```python
from build123d import *

# Parameters (mm, degrees)
SKETCH1_R           = 6.5
SKETCH1_R_2         = 3
BOSS_EXTRUDE1_DEPTH = 5
SKETCH2_R           = 10
BOSS_EXTRUDE2_DEPTH = 10
SKETCH3_W           = 22
SKETCH3_H           = 22
BOSS_EXTRUDE3_DEPTH = 3
FILLET1_R           = 3
SKETCH4_R           = 1.5
CUT_EXTRUDE1_DEPTH  = 3


with BuildPart() as part:
    # Sketch1 → Boss-Extrude1 (new body)
    with BuildSketch(Plane.XY):
        with Locations((-148.746139417, 0)):
            Circle(SKETCH1_R)
        with Locations((-148.746139417, 0)):
            Circle(SKETCH1_R_2, mode=Mode.SUBTRACT)
    extrude(amount=BOSS_EXTRUDE1_DEPTH)

    # Sketch2 → Boss-Extrude2 (add)
    with BuildSketch(Plane.XY.offset(5)):
        with Locations((-148.746139417, 0)):
            Circle(SKETCH2_R)
    extrude(amount=BOSS_EXTRUDE2_DEPTH)

    # Sketch3 → Boss-Extrude3 (add)
    with BuildSketch(Plane.XY.offset(15)):
        with Locations((-148.746139417, 0)):
            Rectangle(SKETCH3_W, SKETCH3_H)
    extrude(amount=BOSS_EXTRUDE3_DEPTH)

    # Fillet1
    fillet1_edges = [part.edges().sort_by_distance(p)[0] for p in [
        (-137.746139417, -11, 16.5),
        (-137.746139417, 11, 16.5),
        (-159.746139417, 11, 16.5),
        (-159.746139417, -11, 16.5),
    ]]
    fillet(fillet1_edges, radius=FILLET1_R)

    # Sketch4 → Cut-Extrude1 (cut)
    with BuildSketch(Plane(origin=(0, 0, 15), x_dir=(-1, 0, 0), z_dir=(0, 0, -1))):
        with Locations((157.446139417, 8.7)):
            Circle(SKETCH4_R)
        with Locations((157.446139417, -8.7)):
            Circle(SKETCH4_R)
        with Locations((140.046139417, -8.7)):
            Circle(SKETCH4_R)
        with Locations((140.046139417, 8.7)):
            Circle(SKETCH4_R)
    extrude(amount=-CUT_EXTRUDE1_DEPTH, mode=Mode.SUBTRACT)


solid = part.part
```
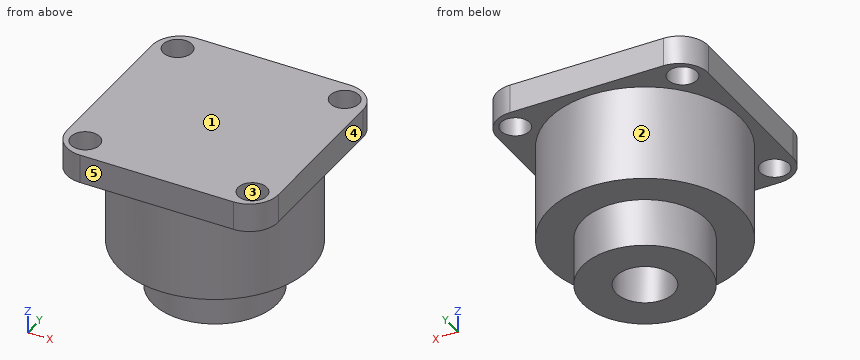
The listing builds one solid part. Answer for the finished solid, in the listing's coordinates (mm). Face numbers are marked on the shaded views. A direction names the side the tool comes from. Coordinates: 2 decimals unless noted, no trailing zeros. Order: outer loops, then holes, each group sorted by start corner. A loop starts at its lowest first (then second) coordinate and runs counter-clockwise, first axis right, second up. Notation, with made-up numbers: M 38,6.5 L 80,6.5 A23 ccw 80,42.5 Z; hole C 18,-3.5 d4. An arc over 180 degrees is marked long. Answer as a JSON object with one key per item and string values. Group by question number.
1. Flat-ended cylindrical pins translate along their axes: P1, Ø2, axis at x = -142, z = 5, coming from the +Y side; P2, Ø5, axis at x = -140.05, y = -8.7, coming from the -Z side; P3, Ø3, axis at x = -155.5, z = 6.5, coming from the -Y side. Find the tip coordinate at first contact, or state that the pin passes through.
2. Determine the mould class of the marked faces 3, 4 and 5 for opening direction Y: released by +Y, released by -Y, zero draft, split by the parting line, or undercut.
3. Section C-C on y = 2 is taken. Write down the section's boundary in (x, z).
4. Section A-A on y = 7.5 is taken. Write down the section's boundary in (x, z).
5. A tool of negligible diameter and unlimited length cuts with its end or side. For the marked faces 1 and 2, from which of +Z, -Z, +X, -X, +Y, -Y can it reach the whole face along a straight path? Write none if from no direction.
6. Section B-B on z = 15.5 is taken. Write down the section's boundary in (x, y).
7. Section D-D on x = -150.25 is taken. Write down the section's boundary in (y, z).
8. Straight lines are drawn through the part: line 1 (Z direction, x = -143.75, y = -10); line 2 (Z direction, x = -158.25, y = 1.5); line 3 (Y direction, x = -139.5, z = 17). For each, find the intervals that lie inside material, in ascending order.
Values follow:
{
 "1": {"P1": "y = 8.18", "P2": "z = 5", "P3": "y = -8.51"},
 "2": {"face 3": "undercut", "face 4": "zero draft", "face 5": "released by -Y"},
 "3": {"outline": "M -159.75,15 L -158.54,15 L -158.54,5 L -154.93,5 L -154.93,0 L -150.98,0 L -150.98,5 L -146.51,5 L -146.51,0 L -142.56,0 L -142.56,5 L -138.95,5 L -138.95,15 L -137.75,15 L -137.75,18 L -159.75,18 Z"},
 "4": {"outline": "M -159.75,15 L -158.35,15 L -158.35,18 L -159.75,18 Z; M -156.55,15 L -155.36,15 L -155.36,5 L -142.13,5 L -142.13,15 L -140.95,15 L -140.95,18 L -156.55,18 Z; M -139.15,15 L -137.75,15 L -137.75,18 L -139.15,18 Z"},
 "5": {"face 1": "+Z, +X, -X, +Y, -Y", "face 2": "-Z"},
 "6": {"outline": "M -159.75,-8 A3 ccw -156.75,-11 L -140.75,-11 A3 ccw -137.75,-8 L -137.75,8 A3 ccw -140.75,11 L -156.75,11 A3 ccw -159.75,8 Z; hole C -157.45,-8.7 d3; hole C -157.45,8.7 d3; hole C -140.05,-8.7 d3; hole C -140.05,8.7 d3"},
 "7": {"outline": "M -11,15 L -9.89,15 L -9.89,5 L -6.32,5 L -6.32,0 L -2.6,0 L -2.6,5 L 2.6,5 L 2.6,0 L 6.32,0 L 6.32,5 L 9.89,5 L 9.89,15 L 11,15 L 11,18 L -11,18 Z"},
 "8": {"line 1": "15 to 18", "line 2": "5 to 18", "line 3": "-10.73 to -10.1, -7.3 to 7.3, 10.1 to 10.73"}
}
